```python
from build123d import *

# Parameters (mm, degrees)
U_FORK_BASE_DEPTH   = 50
U_START             = -50
U_WRAP_LAYER_DEPTH  = 50
WRAP_START          = -4
WRAP_RECESS_1_DEPTH = 4
WRAP_RECESS_2_DEPTH = 4
ARM_PAD_1_DEPTH     = 8
ARM_PAD_2_DEPTH     = 8
ARM_START           = -8
ARM_PAD_3_DEPTH     = 8
ARM_PAD_4_DEPTH     = 8
ARM_PAD_5_DEPTH     = 8
PIN_HOLE_SKETCH_R   = 10
PIN_HOLE_DEPTH      = 70
FACE_RELIEF_1_DEPTH = 1
FACE_START          = -1
FACE_RELIEF_2_DEPTH = 1


with BuildPart() as part:
    # U Fork Profile Sketch → U Fork Base (new body)
    with BuildSketch(Plane.XY):
        with BuildLine():
            ThreePointArc((0, 53), (-23, 30), (0, 7))
            Line((0, 7), (46, 7))
            Line((46, 7), (46, 0))
            Line((46, 0), (0, 0))
            ThreePointArc((0, 0), (-30, 30), (0, 60))
            Line((0, 60), (46, 60))
            Line((46, 60), (46, 53))
            Line((46, 53), (0, 53))
        make_face()
    extrude(amount=U_FORK_BASE_DEPTH)

    # U Wrap Layer Sketch → U Wrap Layer (add)
    with BuildSketch(Plane.XY.offset(50).offset(U_START)):
        with BuildLine():
            Line((0, 53), (46, 53))
            Line((46, 53), (46, 45))
            Line((46, 45), (0, 45))
            ThreePointArc((0, 45), (-15, 30), (0, 15))
            Line((0, 15), (46, 15))
            Line((46, 15), (46, 7))
            Line((46, 7), (0, 7))
            ThreePointArc((0, 7), (-23, 30), (0, 53))
        make_face()
    extrude(amount=U_WRAP_LAYER_DEPTH)

    # Wrap Recess 1 Sketch → Wrap Recess 1 (cut)
    with BuildSketch(Plane.XY.offset(50).offset(WRAP_START)):
        with BuildLine():
            Line((0, 45), (46, 45))
            Line((46, 45), (46, 53))
            Line((46, 53), (0, 53))
            ThreePointArc((0, 53), (-23, 30), (0, 7))
            Line((0, 7), (46, 7))
            Line((46, 7), (46, 15))
            Line((46, 15), (0, 15))
            ThreePointArc((0, 15), (-15, 30), (0, 45))
        make_face()
    extrude(amount=WRAP_RECESS_1_DEPTH, mode=Mode.SUBTRACT)

    # Wrap Recess 2 Sketch → Wrap Recess 2 (cut)
    with BuildSketch(Plane(origin=(0, 0, 0), x_dir=(-1, 0, 0), z_dir=(0, 0, -1))):
        with BuildLine():
            Line((-46, 45), (0, 45))
            ThreePointArc((0, 45), (15, 30), (0, 15))
            Line((0, 15), (-46, 15))
            Line((-46, 15), (-46, 7))
            Line((-46, 7), (0, 7))
            ThreePointArc((0, 7), (23, 30), (0, 53))
            Line((0, 53), (-46, 53))
            Line((-46, 53), (-46, 45))
        make_face()
    extrude(amount=-WRAP_RECESS_2_DEPTH, mode=Mode.SUBTRACT)

    # Arm Pad 1 Sketch → Arm Pad 1 (add)
    with BuildSketch(Plane.XZ.offset(-45)):
        with BuildLine():
            ThreePointArc((46, 10), (61, 25), (46, 40))
            Line((46, 40), (46, 10))
        make_face()
    extrude(amount=-ARM_PAD_1_DEPTH)

    # Arm Pad 2 Sketch → Arm Pad 2 (add)
    with BuildSketch(Plane.XZ.offset(-45)):
        with BuildLine():
            Line((46, 46), (46, 40))
            ThreePointArc((46, 40), (61, 25), (46, 10))
            Line((46, 10), (46, 4))
            ThreePointArc((46, 4), (67, 25), (46, 46))
        make_face()
    extrude(amount=-ARM_PAD_2_DEPTH)

    # Arm Pad 3 Sketch → Arm Pad 3 (add)
    with BuildSketch(Plane(origin=(0, 15, 0), x_dir=(1, 0, 0), z_dir=(0, 1, 0)).offset(ARM_START)):
        with BuildLine():
            ThreePointArc((46, -40), (61, -25), (46, -10))
            Line((46, -10), (46, -40))
        make_face()
        with BuildLine():
            ThreePointArc((46, -46), (67, -25), (46, -4))
            Line((46, -4), (46, -10))
            ThreePointArc((46, -10), (61, -25), (46, -40))
            Line((46, -40), (46, -46))
        make_face()
    extrude(amount=ARM_PAD_3_DEPTH)

    # Arm Pad 4 Sketch → Arm Pad 4 (add)
    with BuildSketch(Plane(origin=(0, 60, 0), x_dir=(1, 0, 0), z_dir=(0, 1, 0)).offset(ARM_START)):
        with BuildLine():
            ThreePointArc((46, -50), (71, -25), (46, 0))
            Line((46, 0), (46, -4))
            ThreePointArc((46, -4), (67, -25), (46, -46))
            Line((46, -46), (46, -50))
        make_face()
        with BuildLine():
            ThreePointArc((46, -46), (67, -25), (46, -4))
            Line((46, -4), (46, -46))
        make_face()
    extrude(amount=ARM_PAD_4_DEPTH)

    # Arm Pad 5 Sketch → Arm Pad 5 (add)
    with BuildSketch(Plane.XZ):
        with BuildLine():
            Line((46, 50), (46, 0))
            ThreePointArc((46, 0), (71, 25), (46, 50))
        make_face()
    extrude(amount=-ARM_PAD_5_DEPTH)

    # Pin Hole Sketch → Pin Hole (cut)
    with BuildSketch(Plane.XZ):
        with Locations(Location((46, 25, 0), (0, 0, 270))):
            Circle(PIN_HOLE_SKETCH_R)
    extrude(amount=-PIN_HOLE_DEPTH, mode=Mode.SUBTRACT)

    # Face Relief 1 Sketch → Face Relief 1 (cut)
    with BuildSketch(Plane.XZ.offset(-52)):
        with BuildLine():
            Line((46, 50), (46, 46))
            ThreePointArc((46, 46), (67, 25), (46, 4))
            Line((46, 4), (46, 0))
            ThreePointArc((46, 0), (71, 25), (46, 50))
        make_face()
    extrude(amount=-FACE_RELIEF_1_DEPTH, mode=Mode.SUBTRACT)

    # Face Relief 2 Sketch → Face Relief 2 (cut)
    with BuildSketch(Plane(origin=(0, 8, 0), x_dir=(1, 0, 0), z_dir=(0, 1, 0)).offset(FACE_START)):
        with BuildLine():
            Line((46, 0), (46, -4))
            ThreePointArc((46, -4), (67, -25), (46, -46))
            Line((46, -46), (46, -50))
            ThreePointArc((46, -50), (71, -25), (46, 0))
        make_face()
    extrude(amount=FACE_RELIEF_2_DEPTH, mode=Mode.SUBTRACT)


solid = part.part
```
Could you check a few things on this model? Use its own coordinates, in mm. A direction names the side the tool comes from. Coordinates: 2 decimals unless noted, no trailing zeros. Write each loop counter-clockwise with the first axis right and the second up, starting at its lowest first coordinate (ties: lowest second). Pieces come first, ordered by that corner, then holes. Notation, with made-up numbers: (45.5, -13.5) -> (50.5, -13.5) arc R29 ccw to (50.5, 13.5) -> close; hole circle Ø11 at (56, 24). An arc over 180 degrees is marked (long way). One line per question, with ' | ' between items. Start each with the question number.
1. If we section it at A-A (x = 28.5): Please give me the cut outline in (y, z), and give its area (3 significant figures).
2. Please list where these lines run through material, in increasing order: line 1 along Y through (x, z) = (20.5, 6.5); line 2 along Y through (x, z) = (9, 2.5); line 3 along X through (y, z) = (3, 25).
3. If we section it at D-D (x = 41): Please give me the cut outline in (y, z), and give its area (3 significant figures).
4. For faces 1 (the face through (26, 45, 25)), 2 (the face through (-22.994, 29.494, 1.972)), 3 (the face through (67, 11, 25)), 4 (the face through (11, 46, 46)), which set-ups out of +Z, -Z, +X, -X, +Y, -Y let a thin tool reach every point of the face, with its end or its side?
5. Will these pins go through, and if not, where does the flat tip stop? P1, Ø23, axis at x = -4.5, y = 22.5, coming from the +Z side; P2, Ø4, axis at x = 57, y = 6, coming from the -Z side; P3, Ø18, axis at x = 46, z = 25, coming from the +Y side; P4, Ø1, axis at y = 49.5, z = 36, coming from the +X side.
6. Thinking about a two-plate mould opening in X: for faces 5 (the face through (-15, 30, 25)), 6 (the face through (-29.993, 29.34, 24.65)), 7 (the face through (37.128, 7.395, 20.386)), 8 (the face through (38, 7, 3)), which applies, pulls with the +X half, pulls with the -X half, needs draft (parallel to the pull), parting line crosses it, or undercut?
7. If we section it at C-C (y = 30): Please give me the cut outline in (x, z).
8. If we section it at B-B (z = 25): Please give me the cut outline in (x, y).
Return value:
1) outline: (0, 0) -> (7, 0) -> (7, 4) -> (15, 4) -> (15, 46) -> (7, 46) -> (7, 50) -> (0, 50) -> close; (45, 4) -> (53, 4) -> (53, 0) -> (60, 0) -> (60, 50) -> (53, 50) -> (53, 46) -> (45, 46) -> close | area: 1,370 mm²
2) line 1: y = 0 to 15, 45 to 60 | line 2: y = 0 to 7, 53 to 60 | line 3: x = -13.08 to 36, 56 to 71
3) outline: (0, 0) -> (7, 0) -> (7, 4) -> (15, 4) -> (15, 16.34) -> (0, 16.34) -> close; (0, 33.66) -> (15, 33.66) -> (15, 46) -> (7, 46) -> (7, 50) -> (0, 50) -> close; (45, 4) -> (53, 4) -> (53, 0) -> (60, 0) -> (60, 16.34) -> (45, 16.34) -> close; (45, 33.66) -> (60, 33.66) -> (60, 50) -> (53, 50) -> (53, 46) -> (45, 46) -> close | area: 852 mm²
4) face 1: +Z, -Z, +X | face 2: -Z, +X | face 3: +X | face 4: +Z, +X
5) P1: stops at z = 46 | P2: stops at z = 1.68 | P3: passes through | P4: stops at x = 64.19
6) face 5: pulls with the +X half | face 6: pulls with the -X half | face 7: undercut | face 8: needs draft
7) outline: (-30, 0) -> (-23, 0) -> (-23, 4) -> (-15, 4) -> (-15, 46) -> (-23, 46) -> (-23, 50) -> (-30, 50) -> close
8) outline: (0, 0) -> (36, 0) -> (36, 15) -> (0, 15) arc R15 cw to (0, 45) -> (36, 45) -> (36, 60) -> (0, 60) arc R30 ccw to start; (56, 0) -> (71, 0) -> (71, 7) -> (67, 7) -> (67, 15) -> (56, 15) -> close; (56, 45) -> (67, 45) -> (67, 53) -> (71, 53) -> (71, 60) -> (56, 60) -> close
